from build123d import *

# Parameters (mm, degrees)
BASE_FLANGE_SKETCH_R         = 3.5
BASE_FLANGE_DEPTH            = 10
LOCATING_PAD_SKETCH_W        = 38
LOCATING_PAD_SKETCH_H        = 10
LOCATING_PAD_DEPTH           = 10
HINGE_BARREL_SKETCH_R        = 15
HINGE_BARREL_SKETCH_R_2      = 6
HINGE_BARREL_DEPTH           = 76.5
HINGE_START                  = 38.5
BARREL_EXTENSION_SKETCH_R    = 15
BARREL_EXTENSION_SKETCH_R_2  = 6
HINGE_BARREL_EXTENSION_DEPTH = 38.5
PIN_BORE_SKETCH_R            = 6
HINGE_PIN_BORE_12_DEPTH      = 115
GUIDE_WALLS_SKETCH_W         = 38.5
GUIDE_WALLS_SKETCH_H         = 70
GUIDE_WALLS_DEPTH            = 10
CENTRE_FIN_DEPTH             = 12
FIN_V_SLOT_SKETCH_W          = 12
FIN_V_SLOT_SKETCH_H          = 11.180339887
FIN_V_SLOT_DEPTH             = 50
FIN_RELIEF_CUT_DEPTH         = 50
THROUGH_BORE_SKETCH_R        = 6
THROUGH_BORE_12_DEPTH        = 200
WALL_WINDOWS_DEPTH           = 4


with BuildPart() as part:
    # Base Flange Sketch → Base Flange (new body)
    with BuildSketch(Plane(origin=(0, 0, 0), x_dir=(1, 0, 0), z_dir=(0, 1, 0))):
        with BuildLine():
            Line((15, -4), (15, -19))
            Line((15, -19), (-15, -19))
            Line((-15, -19), (-15, 19))
            Line((-15, 19), (15, 19))
            Line((15, 19), (15, 4))
            ThreePointArc((15, 4), (11, 0), (15, -4))
        make_face()
        with Locations(Location((3, 10, 0), (0, 0, 270))):
            Circle(BASE_FLANGE_SKETCH_R, mode=Mode.SUBTRACT)
        with Locations(Location((3, -10, 0), (0, 0, 270))):
            Circle(BASE_FLANGE_SKETCH_R, mode=Mode.SUBTRACT)
    extrude(amount=BASE_FLANGE_DEPTH)

    # Locating Pad Sketch → Locating Pad (add)
    with BuildSketch(Plane.ZY.offset(15)):
        with Locations((0, 5)):
            Rectangle(LOCATING_PAD_SKETCH_W, LOCATING_PAD_SKETCH_H)
    extrude(amount=LOCATING_PAD_DEPTH)

    # Hinge Barrel Sketch → Hinge Barrel (add)
    with BuildSketch(Plane.XY.offset(19)):
        with Locations((-30, 5)):
            Circle(HINGE_BARREL_SKETCH_R)
        with Locations((-30, 5)):
            Circle(HINGE_BARREL_SKETCH_R_2, mode=Mode.SUBTRACT)
    extrude(amount=-HINGE_BARREL_DEPTH)

    # Barrel Extension Sketch → Hinge Barrel Extension (add)
    with BuildSketch(Plane.XY.offset(19).offset(HINGE_START)):
        with Locations((-30, 5)):
            Circle(BARREL_EXTENSION_SKETCH_R)
        with Locations((-30, 5)):
            Circle(BARREL_EXTENSION_SKETCH_R_2, mode=Mode.SUBTRACT)
    extrude(amount=-HINGE_BARREL_EXTENSION_DEPTH)

    # Pin Bore Sketch → Hinge Pin Bore Ø12 (cut)
    with BuildSketch(Plane.XY.offset(57.5)):
        with Locations((-30, 5)):
            Circle(PIN_BORE_SKETCH_R)
    extrude(amount=-HINGE_PIN_BORE_12_DEPTH, mode=Mode.SUBTRACT)

    # Guide Walls Sketch → Guide Walls (add, symmetric)
    with BuildSketch(Plane(origin=(-30, 0, 0), x_dir=(0, 0, -1), z_dir=(1, 0, 0))):
        with Locations((38.25, 40)):
            Rectangle(GUIDE_WALLS_SKETCH_W, GUIDE_WALLS_SKETCH_H)
        with Locations((-38.25, 40)):
            Rectangle(GUIDE_WALLS_SKETCH_W, GUIDE_WALLS_SKETCH_H)
    extrude(amount=GUIDE_WALLS_DEPTH, both=True)

    # Centre Fin Sketch → Centre Fin (add)
    with BuildSketch(Plane.ZY.offset(40)):
        with BuildLine():
            Line((-19, 16.180339887), (19, 16.180339887))
            Line((19, 16.180339887), (19, 111.180339887))
            Line((19, 111.180339887), (6, 111.180339887))
            Line((6, 111.180339887), (6, 75))
            ThreePointArc((6, 75), (0, 69), (-6, 75))
            Line((-6, 75), (-6, 111.180339887))
            Line((-6, 111.180339887), (-19, 111.180339887))
            Line((-19, 111.180339887), (-19, 16.180339887))
        make_face()
    extrude(amount=-CENTRE_FIN_DEPTH)

    # Fin V-Slot Sketch → Fin V-Slot (cut)
    with BuildSketch(Plane.XY.offset(19)):
        with Locations((-34, 105.590169944)):
            Rectangle(FIN_V_SLOT_SKETCH_W, FIN_V_SLOT_SKETCH_H)
    extrude(amount=-FIN_V_SLOT_DEPTH, mode=Mode.SUBTRACT)

    # Fin Relief Sketch → Fin Relief Cut (cut)
    with BuildSketch(Plane.XY.offset(19)):
        Polygon((-40, 75), (-28, 100), (-40, 100), align=None)
    extrude(amount=-FIN_RELIEF_CUT_DEPTH, mode=Mode.SUBTRACT)

    # Through Bore Sketch → Through Bore Ø12 (cut)
    with BuildSketch(Plane.XY.offset(57.5)):
        with Locations((-30, 5)):
            Circle(THROUGH_BORE_SKETCH_R)
    extrude(amount=-THROUGH_BORE_12_DEPTH, mode=Mode.SUBTRACT)

    # Wall Window Sketch → Wall Windows (cut, symmetric)
    with BuildSketch(Plane(origin=(-30, 0, 0), x_dir=(0, 0, -1), z_dir=(1, 0, 0))):
        Polygon((57.5, 75), (38.25, 75), (57.5, 45.590169944), align=None)
        Polygon((-57.5, 75), (-57.5, 45.590169944), (-37.5, 75), align=None)
    extrude(amount=WALL_WINDOWS_DEPTH, both=True, mode=Mode.SUBTRACT)


solid = part.part
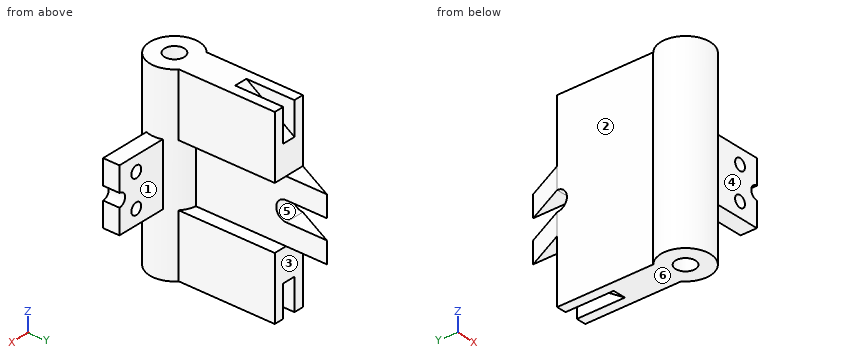
Can you work these out from the model? Positions are in its coordinate system, mm. Face numbers are marked on the shaded views. A direction names the side the tool comes from. Give positions to 0.01 mm unless a question says otherwise; leave off trailing zeros. Write each loop counter-clockwise with the first axis right and the second up, starting at its lowest first coordinate (ties: lowest second). Pieces come first, ordered by that corner, then holes. Notation, with made-up numbers: (19, 27) -> (47, 27) arc R22 ccw to (47, 43) -> close; hole circle Ø3 at (75.25, 7.5). An arc over 180 degrees is marked (long way). Answer as a JSON object with one key per item and string values. Group by question number.
Item 1: We'd pull the mould along Z, two halves only. Please class the marked faces 4, 5 and 6: +Z half, -Z half, draft (parallel to the pull), parting line (faces both ways), or undercut.
Item 2: Suppose I cut it at C-C (x = -30). Please give me the cut outline in (y, z), plus the area to 3 significant figures.
Item 3: I'm going to push flat-ended pins straight in: P1, Ø10, axis at x = -12, z = 22.5, coming from the -Y side; P2, Ø15.5, axis at x = 7, z = -9, coming from the +Y side; P3, Ø11.5, axis at y = 40, z = -6, coming from the +X side. Where does each tip first touch, or does it pass through?
Item 4: For the marked faces 1, 2 and 3, which set-ups out of +Z, -Z, +X, -X, +Y, -Y let a thin tool reach every point of the face, with its end or its side?
Item 5: Please list where these lines run through material, in increasing order: line 1 (X direction, y = 4.5, z = -10); line 2 (X direction, y = 66, z = 53); line 3 (X direction, y = 6, z = 10). Write a range as [from, to].
Item 6: Suppose I cut it at A-A (z = 10). Please give me the cut outline in (x, y).
Item 7: Suppose I cut it at D-D (z = -29.5). Please give me the cut outline in (x, y), plus the area to 3 significant figures.
Item 8: Suppose I cut it at B-B (x = 3). Please give me the cut outline in (y, z).
Findings:
{
 "1": {"face 4": "draft", "face 5": "undercut", "face 6": "-Z half"},
 "2": {"outline": "(-10, -57.5) -> (-1, -57.5) -> (-1, 57.5) -> (-10, 57.5) -> close; (11, -57.5) -> (45.59, -57.5) -> (75, -38.25) -> (75, -19) -> (95.83, -19) -> (95.83, -6) -> (75, -6) arc R6 cw to (75, 6) -> (95.83, 6) -> (95.83, 19) -> (75, 19) -> (75, 37.5) -> (45.59, 57.5) -> (11, 57.5) -> close", "area": "8,300 mm²"},
 "3": {"P1": "stops at y = -2.48", "P2": "stops at y = 10", "P3": "stops at x = -28"},
 "4": {"face 1": "+Z, -Z, +X, +Y", "face 2": "+Z, -Z, -X, +Y", "face 3": "-Z, +X, -X, +Y"},
 "5": {"line 1": "x = [-44.99, -35.98], [-24.02, -0.5], [6.5, 15]", "line 2": "x = [-40, -34], [-26, -20]", "line 3": "x = [-44.97, -35.92], [-24.08, -0.5], [6.5, 15]"},
 "6": {"outline": "(-40, 16.18) arc R15 ccw (long way) to (-15.86, 0) -> (-0.5, 0) -> (-0.5, 10) -> (-15.86, 10) arc R15 ccw to (-28, 19.87) -> (-28, 100) -> (-40, 75) -> close; (6.5, 0) -> (15, 0) -> (15, 10) -> (6.5, 10) -> close; hole circle Ø12 at (-30, 5)"},
 "7": {"outline": "(-40, 16.18) arc R15 ccw (long way) to (-20, 16.18) -> (-20, 75) -> (-40, 75) -> close; hole circle Ø12 at (-30, 5)", "area": "1,720 mm²"},
 "8": {"outline": "(0, -19) -> (10, -19) -> (10, -13.5) -> (0, -13.5) -> close; (0, -6.5) -> (10, -6.5) -> (10, 6.5) -> (0, 6.5) -> close; (0, 13.5) -> (10, 13.5) -> (10, 19) -> (0, 19) -> close"}
}
